from build123d import *

# Parameters (mm, degrees)
KEYWAY_1_SKETCH_W  = 42
KEYWAY_1_SKETCH_H  = 8
KEYWAY_1_CUT_DEPTH = 4
KEYWAY_2_SKETCH_W  = 32
KEYWAY_2_SKETCH_H  = 8
KEYWAY_2_CUT_DEPTH = 4


with BuildPart() as part:
    # Shaft Profile Sketch → Stepped Shaft Body (revolve)
    with BuildSketch(Plane.XY, mode=Mode.PRIVATE) as stepped_shaft_body_sk:
        Polygon((0, 0), (0, 12), (42, 12), (42, 15), (120, 15), (120, 16), (128, 16), (128, 15), (190, 15), (190, 14), (245.5, 14), (245.5, 12.5), (247, 12.5), (247, 14), (250, 14), (250, 0), align=None)
    revolve(stepped_shaft_body_sk.sketch.rotate(Axis((0, 0, 0), (1, 0, 0)), 90), axis=Axis((0, 0, 0), (1, 0, 0)))

    # Keyway 1 Sketch → Keyway 1 Cut (cut)
    with BuildSketch(Plane(origin=(0, 12, 0), x_dir=(1, 0, 0), z_dir=(0, 1, 0))):
        with Locations((21, 0)):
            Rectangle(KEYWAY_1_SKETCH_W, KEYWAY_1_SKETCH_H)
    extrude(amount=-KEYWAY_1_CUT_DEPTH, mode=Mode.SUBTRACT)

    # Keyway 2 Sketch → Keyway 2 Cut (cut)
    with BuildSketch(Plane(origin=(0, 14, 0), x_dir=(1, 0, 0), z_dir=(0, 1, 0))):
        with Locations((214.5, 0)):
            Rectangle(KEYWAY_2_SKETCH_W, KEYWAY_2_SKETCH_H)
    extrude(amount=-KEYWAY_2_CUT_DEPTH, mode=Mode.SUBTRACT)


solid = part.part
The listing builds one solid part. Answer for the finished solid, in the listing's coordinates (mm). A direction names the side the tool comes from. Round coordinates to 2 decimals unless told otherwise and drop trailing zeros. Order: outer loops, then holes, each group sorted by start corner. A loop starts at its lowest first (then second) coordinate and runs counter-clockwise, first axis right, second up. Notation, with made-up numbers: (59, -7) -> (88, -7) arc R31 ccw to (88, 23) -> close; hole circle Ø8 at (59, 46.5). An arc over 180 degrees is marked (long way). Write each question's results on one line, items separated by ' | '. Start each with the question number.
Q1. Find section B-B (y = 0). Determine the outline of the cut face in (x, z).
Q2. Straight lines are drawn through the part: probe 1 along X at (y, z) = (4, 12); probe 2 along Z at (x, y) = (140.5, 1); probe 3 along Z at (x, y) = (237, 0.5). For each, find the intervals that lie inside material, in ascending order. Write a range as from..to.
Q3. Each of these flat-tipped pins is pushed along its axis until it touches: pin 1 (15 mm diameter, centred on y = 7, z = -0.5, fed in from -X); pin 2 (6.5 mm diameter, centred on x = 214.5, z = -2, fed in from +Y); pin 3 (1.5 mm diameter, centred on x = 27, y = -5, fed in from +Z); pin 4 (3 mm diameter, centred on x = 75, z = 0.5, fed in from +Y). Where does it stop, or does it pass through?
Q4. Which of the six approach directions +Z, -Z, +X, -X, +Y, -Y give full straight-line access (tool end or side, diameter ignored) to faces 5 (the flat face through (21, 8, 0)), 6 (the cylindrical face through (159.43, -12.65, 8.06)), 7 (the cylindrical face through (21, -12, 0)), 8 (the cylindrical face through (246.26, -3.755, 11.923)), 9 (the flat face through (214, 10, 0))?
Q5. Find section C-C (x = 222). Determine the outline of the cut face in (y, z), then the cut area to 3 significant figures.
Q6. The mould has two halves that part along X. Classify faces 1 (the flat face through (247, -11.5, 5.3)), 2 (the cylindrical face through (248.5, 12.4, 6.5)), 3 (the flat face through (250, 0, 0)), 4 (the flat face through (0, -1, 0)): pulls with the +X half, pulls with the -X half, needs draft (parallel to the pull), parting line crosses it, or undercut.
Q7. Find section D-D (z = -9.5). Determine the outline of the cut face in (x, y).
Worked answers:
1) outline: (0, -12) -> (42, -12) -> (42, -15) -> (120, -15) -> (120, -16) -> (128, -16) -> (128, -15) -> (190, -15) -> (190, -14) -> (245.5, -14) -> (245.5, -12.5) -> (247, -12.5) -> (247, -14) -> (250, -14) -> (250, 14) -> (247, 14) -> (247, 12.5) -> (245.5, 12.5) -> (245.5, 14) -> (190, 14) -> (190, 15) -> (128, 15) -> (128, 16) -> (120, 16) -> (120, 15) -> (42, 15) -> (42, 12) -> (0, 12) -> close
2) probe 1: x = 42..245.5, 247..250 | probe 2: z = -14.97..14.97 | probe 3: z = -13.99..13.99
3) pin 1: stops at x = 0 | pin 2: stops at y = 13.42 | pin 3: stops at z = 11.22 | pin 4: stops at y = 15
4) face 5: -X, +Y | face 6: +X | face 7: -X | face 8: none | face 9: +Y
5) outline: (10, -4) -> (10, 4) -> (13.42, 4) arc R14 ccw (long way) to (13.42, -4) -> close | area: 585 mm2
6) face 1: undercut | face 2: needs draft | face 3: pulls with the +X half | face 4: pulls with the -X half
7) outline: (0, -7.33) -> (42, -7.33) -> (42, -11.61) -> (120, -11.61) -> (120, -12.87) -> (128, -12.87) -> (128, -11.61) -> (190, -11.61) -> (190, -10.28) -> (245.5, -10.28) -> (245.5, -8.12) -> (247, -8.12) -> (247, -10.28) -> (250, -10.28) -> (250, 10.28) -> (247, 10.28) -> (247, 8.12) -> (245.5, 8.12) -> (245.5, 10.28) -> (190, 10.28) -> (190, 11.61) -> (128, 11.61) -> (128, 12.87) -> (120, 12.87) -> (120, 11.61) -> (42, 11.61) -> (42, 7.33) -> (0, 7.33) -> close
